from build123d import *

# Parameters (mm, degrees)
EXTRUDE_1_DEPTH = 8


with BuildPart() as part:
    # 草图1 → 旋转1 (revolve)
    with BuildSketch(Plane.XY, mode=Mode.PRIVATE) as revolve_1_sk:
        Polygon((-13.9, 0), (-14.1, 0), (-16, 1.9), (-16, 7), (-18, 7), (-18, 14.464101615), (-16, 15), (-13.9, 15), (-12, 13.1), (-12, 1.9), align=None)
    revolve(revolve_1_sk.sketch.rotate(Axis((0, 0, 0), (0, -1, 0)), 270), axis=Axis((0, 0, 0), (0, -1, 0)))

    # 草图2 → 拉伸1 (add)
    with BuildSketch(Plane(origin=(0, 15, 0), x_dir=(1, 0, 0), z_dir=(0, 1, 0))):
        Polygon((18, -10.392304845), (18, 10.392304845), (0, 20.784609691), (-18, 10.392304845), (-18, -10.392304845), (0, -20.784609691), align=None)
    extrude(amount=-EXTRUDE_1_DEPTH)

    # 草图3 → 切除-旋转2 (revolve, cut)
    with BuildSketch(Plane.XY, mode=Mode.PRIVATE) as cut_revolve_2_sk:
        Polygon((-29.9, 11.275506225), (-16, 15), (-29.9, 15), align=None)
        Polygon((-13.9, 15), (-12, 13.1), (-12, 0), (0, 0), (0, 15), align=None)
    revolve(cut_revolve_2_sk.sketch.rotate(Axis((0, 0, 0), (0, -1, 0)), 270), axis=Axis((0, 0, 0), (0, -1, 0)), mode=Mode.SUBTRACT)


solid = part.part
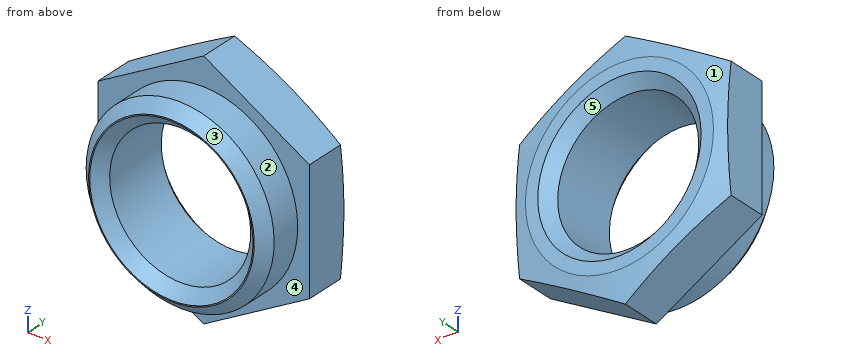
Geometry: final body of the model. Coordinates: model frame, mm. Face numbers are marked on the shaded views. A direction names the side the tool comes from. Coordinates: 2 decimals unless noted, no trailing zeros. Order: outer loops, then holes, each group sorted by start corner. A loop starts at its lowest first (then second) coordinate and runs counter-clockwise, first axis right, second up.
(1) Draft query along X for the marked faces 3, 4 and 5. Return one class per face: pulls with the +X half, pulls with the -X half, needs draft (parallel to the pull), parting line crosses it, or undercut.
(2) Section query C-C (y = 2.75). Return the cut outline in (x, z), plus the area to 3 significant figures.
(3) Section query A-A (z = 0). Return the cut outline in (x, y), plus the area to 3 significant figures.
(4) Access query for the marked faces 1 and 2. Directions: +Z, -Z, +X, -X, +Y, -Y. A direction counts if a zero-diameter tool reaches every point of the face in a straight line with its end or side. Return the directions, or none.
(5) Section query B-B (y = 8.25). Return the cut outline in (x, z), plus the area to 3 significant figures.
(6) Material intervals for probe 1 along X at (y, z) = (8, 0); probe 2 along X at (y, z) = (6.5, 0); probe 3 along Z at (x, y) = (3, 11), sorted ascending.
(7) First-contact query: pin 1 (6 mm diameter, centred on x = 5, z = 16.5, fed in from -Y); pin 2 (3 mm diameter, centred on x = 7.5, y = 7.5, fed in from -Z); pin 3 (10 mm diameter, centred on x = 1, z = 7.5, fed in from -Y); pin 4 (12 mm diameter, centred on x = 13.5, z = 2, fed in from -Y). Flat tips, straight axial feed; report the tip coordinate or a pass-through.
Solution:
1. face 3: parting line crosses it
1. face 4: needs draft
1. face 5: undercut
2. outline: circle Ø32 at (0, 0); hole circle Ø24 at (0, 0)
2. area: 352 mm2
3. outline: (-18, 7) - (-16, 7) - (-16, 1.9) - (-14.1, 0) - (-13.9, 0) - (-12, 1.9) - (-12, 13.1) - (-13.9, 15) - (-16, 15) - (-18, 14.46) - close; (12, 1.9) - (13.9, 0) - (14.1, 0) - (16, 1.9) - (16, 7) - (18, 7) - (18, 14.46) - (16, 15) - (13.9, 15) - (12, 13.1) - close
3. area: 140 mm2
4. face 1: +Y
4. face 2: -Y
5. outline: (-18, -10.39) - (0, -20.78) - (18, -10.39) - (18, 10.39) - (0, 20.78) - (-18, 10.39) - close; hole circle Ø24 at (0, 0)
5. area: 670 mm2
6. probe 1: x = -18 to -12, 12 to 18
6. probe 2: x = -16 to -12, 12 to 16
6. probe 3: z = -19.05 to -11.62, 11.62 to 19.05
7. pin 1: stops at y = 0.14
7. pin 2: stops at z = -17.32
7. pin 3: stops at y = 1.33
7. pin 4: stops at y = 0
